from build123d import *

# Parameters (mm, degrees)
STEPPED_TAB_PLATE_0_5MM_DEPTH = 0.5
CORNER_CHAMFER_0_2X45_A_SIZE  = 0.2
CORNER_CHAMFER_0_2X45_B_SIZE  = 0.2
SCREW_HOLES_SKETCH_R          = 0.2
SCREW_HOLES_2X_DEPTH          = 1
HOLE_GRID_SKETCH_R            = 0.15
HOLE_GRID_3X3_DEPTH           = 1


with BuildPart() as part:
    # Stepped Tab Profile Sketch → Stepped Tab Plate 0.5mm (new body)
    with BuildSketch(Plane.XY):
        with BuildLine():
            ThreePointArc((3.75, 1.5), (3.926776695, 1.573223305), (4, 1.75))
            Line((4, 1.75), (4, 2))
            Line((4, 2), (7.5, 2))
            Line((7.5, 2), (7.5, 0))
            Line((7.5, 0), (0, 0))
            Line((0, 0), (0, 1.5))
            Line((0, 1.5), (3.75, 1.5))
        make_face()
        with BuildLine():
            ThreePointArc((4, -1.75), (3.926776695, -1.573223305), (3.75, -1.5))
            Line((3.75, -1.5), (0, -1.5))
            Line((0, -1.5), (0, 0))
            Line((0, 0), (7.5, 0))
            Line((7.5, 0), (7.5, -2))
            Line((7.5, -2), (4, -2))
            Line((4, -2), (4, -1.75))
        make_face()
    extrude(amount=STEPPED_TAB_PLATE_0_5MM_DEPTH)

    # Corner Chamfer 0.2x45 A
    corner_chamfer_0_2x45_a_edges = [part.edges().sort_by_distance(p)[0] for p in [
        (7.5, 2, 0.25),
        (0, 1.5, 0.25),
    ]]
    chamfer(corner_chamfer_0_2x45_a_edges, length=CORNER_CHAMFER_0_2X45_A_SIZE)

    # Corner Chamfer 0.2x45 B
    corner_chamfer_0_2x45_b_edges = [part.edges().sort_by_distance(p)[0] for p in [
        (7.5, -2, 0.25),
        (0, -1.5, 0.25),
    ]]
    chamfer(corner_chamfer_0_2x45_b_edges, length=CORNER_CHAMFER_0_2X45_B_SIZE)

    # Screw Holes Sketch → Screw Holes 2x (cut)
    with BuildSketch(Plane.XY.offset(0.5)):
        with Locations((2, 0.82)):
            Circle(SCREW_HOLES_SKETCH_R)
        with Locations((2, -0.82)):
            Circle(SCREW_HOLES_SKETCH_R)
    extrude(amount=-SCREW_HOLES_2X_DEPTH, mode=Mode.SUBTRACT)

    # Hole Grid Sketch → Hole Grid 3x3 (cut)
    with BuildSketch(Plane.XY.offset(0.5)):
        with Locations((4.75, 1.25)):
            Circle(HOLE_GRID_SKETCH_R)
        with Locations((5.75, 1.25)):
            Circle(HOLE_GRID_SKETCH_R)
        with Locations((6.75, 1.25)):
            Circle(HOLE_GRID_SKETCH_R)
        with Locations((6.75, 0)):
            Circle(HOLE_GRID_SKETCH_R)
        with Locations((6.75, -1.25)):
            Circle(HOLE_GRID_SKETCH_R)
        with Locations((5.75, -1.25)):
            Circle(HOLE_GRID_SKETCH_R)
        with Locations((4.75, -1.25)):
            Circle(HOLE_GRID_SKETCH_R)
        with Locations((4.75, 0)):
            Circle(HOLE_GRID_SKETCH_R)
        with Locations((5.75, 0)):
            Circle(HOLE_GRID_SKETCH_R)
    extrude(amount=-HOLE_GRID_3X3_DEPTH, mode=Mode.SUBTRACT)


solid = part.part
Design review of the part built by this model. Coordinates are the model's own, in mm. Coordinates: 2 decimals unless noted, no trailing zeros. Order: outer loops, then holes, each group sorted by start corner. A loop starts at its lowest first (then second) coordinate and runs counter-clockwise, first axis right, second up. Notation, with made-up numbers: M 16.5,45 L 30.5,45 A29 cw 30.5,69 Z; hole C 11,1.5 d11. An arc over 180 degrees is marked long. Use a Markdown table: item, result.
(1) Add section B-B (x = 4.75). Give the boundary of the cut face in (y, z).
Worked answers:
| item | result |
|---|---|
| outline | M -2,0 L -1.4,0 L -1.4,0.5 L -2,0.5 Z; M -1.1,0 L -0.15,0 L -0.15,0.5 L -1.1,0.5 Z; M 0.15,0 L 1.1,0 L 1.1,0.5 L 0.15,0.5 Z; M 1.4,0 L 2,0 L 2,0.5 L 1.4,0.5 Z |
(2) Add section C-C (x = 2). Give the boundary of the cut face in (y, z), then the cut area to 3 significant figures.
Worked answers:
| item | result |
|---|---|
| outline | M -1.5,0 L -1.02,0 L -1.02,0.5 L -1.5,0.5 Z; M -0.62,0 L 0.62,0 L 0.62,0.5 L -0.62,0.5 Z; M 1.02,0 L 1.5,0 L 1.5,0.5 L 1.02,0.5 Z |
| area | 1.10 mm2 |
(3) Add section A-A (y = -0.82). Give the boundary of the cut face in (x, z), then the cut area to 3 significant figures.
Worked answers:
| item | result |
|---|---|
| outline | M 0,0 L 1.8,0 L 1.8,0.5 L 0,0.5 Z; M 2.2,0 L 7.5,0 L 7.5,0.5 L 2.2,0.5 Z |
| area | 3.55 mm2 |
(4) Wall thickness on probe 1 along Y at (x, z) = (2, 0.3); probe 2 along Y at (x, z) = (6.75, 0.3); probe 3 along Y at (x, z) = (2.5, 0.05): over which ranges is each line inside the solid? List them lowest first.
Worked answers:
| item | result |
|---|---|
| probe 1 | y = -1.5 to -1.02, -0.62 to 0.62, 1.02 to 1.5 |
| probe 2 | y = -2 to -1.4, -1.1 to -0.15, 0.15 to 1.1, 1.4 to 2 |
| probe 3 | y = -1.5 to 1.5 |
(5) Add section D-D (z = 0.2). Count the separate pieces of the cut face and the enclosed holes in it, then the cut area to 3 significant figures.
Worked answers:
| item | result |
|---|---|
| separate pieces | 1 |
| enclosed holes | 11 |
| area | 25.1 mm2 |
